Can you work these out from the model? Positions are in its coordinate system, mm. A direction names the side the tool comes from. Round coordinates to 2 decimals unless told otherwise and drop trailing zeros. Order: outer loops, then holes, each group sorted by start corner. A loop starts at its lowest first (then second) coordinate and runs counter-clockwise, first axis right, second up. Notation, with made-up numbers: M 73,-31.75 L 92,-31.75 A24 cw 92,-14.75 Z; hole C 3.5,44.25 d1. An arc over 180 degrees is marked long. Answer as a JSON object with one key per item and string values. Group by question number.
from build123d import *

# Parameters (mm, degrees)
EXTRUDE_1_DEPTH        = 1230
HOLE_WIZARD_6_0_6_1_D  = 6
PATTERN_LINEAR_1_COUNT = 3
PATTERN_LINEAR_1_PITCH = 410


with BuildPart() as part:
    # 草图1 → 拉伸1 (new body)
    with BuildSketch(Plane.XY):
        with BuildLine():
            Line((0, 0), (0, 40))
            Line((0, 40), (3.99, 40))
            ThreePointArc((3.99, 40), (3.997071068, 39.997071068), (4, 39.99))
            Line((4, 39.99), (4, 8.5))
            ThreePointArc((4, 8.5), (5.318019485, 5.318019485), (8.5, 4))
            Line((8.5, 4), (39.99, 4))
            ThreePointArc((39.99, 4), (39.997071068, 3.997071068), (40, 3.99))
            Line((40, 3.99), (40, 0))
            Line((40, 0), (0, 0))
        make_face()
    extrude(amount=EXTRUDE_1_DEPTH)

    # Ø6.0 (6) 直径孔1 (through all)
    with Locations(Plane(origin=(0, 0, 0), x_dir=(-1, 0, 0), z_dir=(0, -1, 0))):
        with Locations((-25, -205)):
            hole_wizard_6_0_6_1 = Hole(HOLE_WIZARD_6_0_6_1_D / 2)

    # 阵列(线性)1: Ø6.0 (6) 直径孔1 ×3
    with Locations(*[(0, 0, i * PATTERN_LINEAR_1_PITCH) for i in range(1, PATTERN_LINEAR_1_COUNT)]):
        add(hole_wizard_6_0_6_1, mode=Mode.SUBTRACT)


solid = part.part
Item 1: I'm going to push flat-ended pins straight in: pin 1 Ø7 at (x, z) = (25, 1025) entering from +Y; pin 2 Ø10 at (y, z) = (8.5, 125.5) entering from +X; pin 3 Ø3.5 at (x, z) = (25, 615) entering from -Y; pin 4 Ø15.5 at (y, z) = (31.5, 545.5) entering from +X. Where does each tip first touch, or does it pass through?
Item 2: On a 3-axis mill with a long thin cutter (end or side, diameter ignored), from which of +Z, -Z, +X, -X, +Y, -Y can I reach the whole of each face in a straight line? I mean faces 1 (the face through (12.7, 3.8, 1230)), 2 (the face through (24, 4, 606)). Say none if no direction works.
Item 3: Suppose I cut it at B-B, the plane y = 15.5. Write out the boundary of the cut face in (x, z), and give its area (3 significant figures).
Item 4: I need wall thicknesses on line 1 (Z direction, x = 25, y = 2.55); line 2 (X direction, y = 1.55, z = 1025); line 3 (Y direction, x = 33, z = 1065). Which ranges of each line are inside material? Lowest first, please.
Computed:
{
 "1": {"pin 1": "stops at y = 4", "pin 2": "stops at x = 40", "pin 3": "passes through", "pin 4": "stops at x = 4"},
 "2": {"face 1": "+Z, +X, -X, +Y, -Y", "face 2": "+Z, -Z, +X, +Y"},
 "3": {"outline": "M 0,0 L 4,0 L 4,1230 L 0,1230 Z", "area": "4,920 mm^2"},
 "4": {"line 1": "z = 0 to 202, 208 to 612, 618 to 1022, 1028 to 1230", "line 2": "x = 0 to 22, 28 to 40", "line 3": "y = 0 to 4"}
}
